from build123d import *

# Parameters (mm, degrees)
SKETCH_1_W             = 125
SKETCH_1_H             = 20
EXTRUDE_1_DEPTH        = 12
CUT_EXTRUDE_1_DEPTH    = 65.422433981
HOLE_WIZARD_M5_1_D     = 4.2
HOLE_WIZARD_M5_1_DEPTH = 10
HOLE_WIZARD_M5_1_TIP   = 1.2618073
CHAMFER_1_SIZE         = 2
CHAMFER_2_SIZE         = 1


with BuildPart() as part:
    # 草图1 → 凸台-拉伸1 (new body)
    with BuildSketch(Plane.XY):
        Rectangle(SKETCH_1_W, SKETCH_1_H)
    extrude(amount=EXTRUDE_1_DEPTH)

    # 草图2 → 切除-拉伸1 (cut, through all)
    with BuildSketch(Plane.XY.offset(12)):
        with BuildLine():
            Line((-45, 3.3), (45, 3.3))
            ThreePointArc((45, 3.3), (48.3, 0), (45, -3.3))
            Line((45, -3.3), (-45, -3.3))
            ThreePointArc((-45, -3.3), (-48.3, 0), (-45, 3.3))
        make_face()
    extrude(amount=-CUT_EXTRUDE_1_DEPTH, mode=Mode.SUBTRACT)

    # M5 螺纹孔1
    with Locations(Plane(origin=(0, -10, 0), x_dir=(-1, 0, 0), z_dir=(0, -1, 0))):
        with Locations((55, -6), (0, -6), (-55, -6)):
            Hole(HOLE_WIZARD_M5_1_D / 2, depth=HOLE_WIZARD_M5_1_DEPTH)
            with Locations((0, 0, -(HOLE_WIZARD_M5_1_DEPTH + HOLE_WIZARD_M5_1_TIP / 2))):  # 118° drill point
                Cone(0, HOLE_WIZARD_M5_1_D / 2, HOLE_WIZARD_M5_1_TIP, mode=Mode.SUBTRACT)

    # 倒角1
    chamfer_1_edges = [part.edges().sort_by_distance(p)[0] for p in [
        (-62.5, 10, 6),
        (62.5, 10, 6),
    ]]
    chamfer(chamfer_1_edges, length=CHAMFER_1_SIZE)

    # 倒角2
    chamfer_2_edges = [part.edges().sort_by_distance(p)[0] for p in [
        (62.5, -10, 6),
        (-62.5, -10, 6),
    ]]
    chamfer(chamfer_2_edges, length=CHAMFER_2_SIZE)


solid = part.part
Model file for the job. Use its own axes, mm. A direction names the side the tool comes from. Round coordinates to 2 decimals unless told otherwise and drop trailing zeros. Loops run counter-clockwise (first coordinate to the right, second up) from the corner with the lowest first, then second, coordinate; pieces in that order, holes last.
1. Tool access for faces 1 (the cylindrical face through (56.94, -4.93, 6.8)), 2 (the flat face through (61.5, 9, 5.9)), 3 (the cylindrical face through (-48.3, -0.1, 6.1)): list every direction of +Z, -Z, +X, -X, +Y, -Y with a clear straight run to the whole face (end or side of a thin tool).
Check values:
face 1: -Y
face 2: +Z, -Z, +X, +Y
face 3: +Z, -Z
2. Band-saw the part on A-A, the plane y = -1.75. List the corners of the cut face in (x, z).
Check values:
outline: (-62.5, 0) - (-47.8, 0) - (-47.8, 12) - (-62.5, 12) - close; (47.8, 0) - (62.5, 0) - (62.5, 12) - (47.8, 12) - close; hole circle Ø4.2 at (-55, 6); hole circle Ø4.2 at (55, 6)
3. Wall check: probe 1 along X at (y, z) = (-7, 5.75); probe 2 along Z at (x, y) = (-55, -4.25); probe 3 along Y at (x, z) = (-2, 1.5). Give the ranges that are in metal, low to high.
Check values:
probe 1: x = -62.5 to -57.09, -52.91 to -2.09, 2.09 to 52.91, 57.09 to 62.5
probe 2: z = 0 to 3.9, 8.1 to 12
probe 3: y = -10 to -3.3, 3.3 to 10
4. Drop flat-ended pins along their axis: P1, Ø10, axis at x = 39, y = 0.5, coming from the +Z side; P2, Ø3.5, axis at x = 55, z = 6, coming from the -Y side. Give the stop position or say it passes through.
Check values:
P1: stops at z = 12
P2: stops at y = 0.21
5. Band-saw the part on B-B, the plane z = 9.5. List the corners of the cut face in (x, y).
Check values:
outline: (-62.5, -9) - (-61.5, -10) - (61.5, -10) - (62.5, -9) - (62.5, 8) - (60.5, 10) - (-60.5, 10) - (-62.5, 8) - close; hole (-45, -3.3) - (45, -3.3) arc R3.3 ccw to (45, 3.3) - (-45, 3.3) arc R3.3 ccw to start
6. Band-saw the part on C-C, the plane x = 31.5. List the corners of the cut face in (y, z), and give its area (3 significant figures).
Check values:
outline: (-10, 0) - (-3.3, 0) - (-3.3, 12) - (-10, 12) - close; (3.3, 0) - (10, 0) - (10, 12) - (3.3, 12) - close
area: 161 mm2
7. Mould opens along X. For faces 4 (the flat face through (1, -3.3, 9)), 5 (the flat face through (-1, 5, 0)), 6 (the flat face through (-61.5, 9, 5.9)), 7 (the cylindrical face through (-53.06, -4.93, 6.8)) say: +X half, -X half, draft (parallel to the pull), parting line (faces both ways), or undercut.
Check values:
face 4: undercut
face 5: draft
face 6: -X half
face 7: undercut
